from build123d import *

# Parameters (mm, degrees)
SKETCH_1_R          = 20
EXTRUDE_1_DEPTH     = 342.5
SKETCH_2_R          = 18
EXTRUDE_2_DEPTH     = 48
SKETCH_3_R          = 17.5
EXTRUDE_3_DEPTH     = 40
EXTRUDE_START       = 48
SKETCH_4_R          = 18
EXTRUDE_4_DEPTH     = 48
EXTRUDE_START_2     = 40
SKETCH_5_R          = 17.5
EXTRUDE_5_DEPTH     = 40
CUT_EXTRUDE_1_DEPTH = 5.71
CHAMFER_1_SIZE      = 2


with BuildPart() as part:
    # 草图1 → 凸台-拉伸1 (new, symmetric)
    with BuildSketch(Plane(origin=(0, 0, 0), x_dir=(0, 0, -1), z_dir=(1, 0, 0))):
        Circle(SKETCH_1_R)
    extrude(amount=EXTRUDE_1_DEPTH, both=True)

    # 草图2 → 凸台-拉伸2 (add)
    with BuildSketch(Plane.ZY.offset(342.5)):
        with Locations(Location((0, 0, 0), (0, 0, 180))):
            Circle(SKETCH_2_R)
    extrude(amount=EXTRUDE_2_DEPTH)

    # 草图3 → 凸台-拉伸3 (add)
    with BuildSketch(Plane.ZY.offset(390.5)):
        Circle(SKETCH_3_R)
    extrude(amount=EXTRUDE_3_DEPTH)

    # 草图4 → 凸台-拉伸4 (add)
    with BuildSketch(Plane(origin=(342.5, 0, 0), x_dir=(0, 0, -1), z_dir=(1, 0, 0)).offset(EXTRUDE_START)):
        Circle(SKETCH_4_R)
    extrude(amount=-EXTRUDE_4_DEPTH)

    # 草图5 → 凸台-拉伸5 (add)
    with BuildSketch(Plane(origin=(390.5, 0, 0), x_dir=(0, 0, -1), z_dir=(1, 0, 0)).offset(EXTRUDE_START_2)):
        with Locations(Location((0, 0, 0), (0, 0, 180))):
            Circle(SKETCH_5_R)
    extrude(amount=-EXTRUDE_5_DEPTH)

    # 草图7 → 切除-拉伸1 (cut)
    with BuildSketch(Plane(origin=(0, 18, 0), x_dir=(1, 0, 0), z_dir=(0, 1, 0))):
        with BuildLine():
            Line((351.5, 5), (381.5, 5))
            ThreePointArc((381.5, 5), (386.5, 0), (381.5, -5))
            Line((381.5, -5), (351.5, -5))
            ThreePointArc((351.5, -5), (346.5, 0), (351.5, 5))
        make_face()
        with BuildLine():
            Line((-351.5, -5), (-381.5, -5))
            ThreePointArc((-381.5, -5), (-386.5, 0), (-381.5, 5))
            Line((-381.5, 5), (-351.5, 5))
            ThreePointArc((-351.5, 5), (-346.5, 0), (-351.5, -5))
        make_face()
    extrude(amount=-CUT_EXTRUDE_1_DEPTH, mode=Mode.SUBTRACT)

    # 倒角1
    chamfer_1_edges = [part.edges().sort_by_distance(p)[0] for p in [
        (-430.5, 0, -17.5),
        (430.5, 0, -17.5),
    ]]
    chamfer(chamfer_1_edges, length=CHAMFER_1_SIZE)


solid = part.part
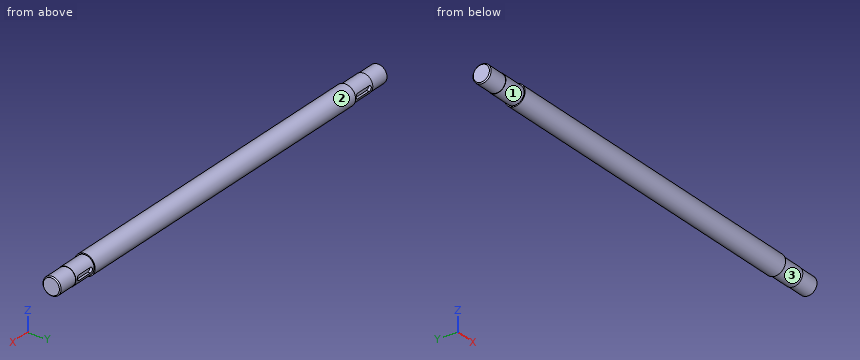
Verification items for the finished model (mm, model axes). Face numbers are marked on the shaded views. A direction names the side the tool comes from. Give positions to 0.01 mm unless a question says otherwise; leave off trailing zeros. Write each loop counter-clockwise with the first axis right and the second up, starting at its lowest first coordinate (ties: lowest second). Pieces come first, ordered by that corner, then holes.
(1) Gauge pin test, flat ends, axial feed: pin 1 (5 mm diameter, centred on x = 372, z = -2, fed in from +Y); pin 2 (1.5 mm diameter, centred on x = 211, z = -9.5, fed in from +Y); pin 3 (4 mm diameter, centred on x = -366.5, y = 15, fed in from +Z). Record the tip position at first contact, or that the pin passes through.
(2) Access from +Z, -Z, +X, -X, +Y, -Y to the whole of each face (thin tool, end or side, straight path). Record for the marked faces 1, 2 and 3.
(3) Cross-section at A-A (y = 0). Enter the section's corners in (x, z), plus the area to 3 significant figures.
(4) Cross-section at B-B (x = 303). Enter the section's corners in (y, z).
(5) Material ranges on line 1 (X direction, y = -14, z = -13.5); line 2 (Y direction, x = 384, z = 4.5); line 3 (Z direction, x = 316, y = 0.5), recorded low to high.
Worked out:
1. pin 1: stops at y = 12.29
1. pin 2: stops at y = 17.98
1. pin 3: stops at z = 12.45
2. face 1: -X
2. face 2: +X, -X
2. face 3: +X
3. outline: (-430.5, -15.5) - (-428.5, -17.5) - (-390.5, -17.5) - (-390.5, -18) - (-342.5, -18) - (-342.5, -20) - (342.5, -20) - (342.5, -18) - (390.5, -18) - (390.5, -17.5) - (428.5, -17.5) - (430.5, -15.5) - (430.5, 15.5) - (428.5, 17.5) - (390.5, 17.5) - (390.5, 18) - (342.5, 18) - (342.5, 20) - (-342.5, 20) - (-342.5, 18) - (-390.5, 18) - (-390.5, 17.5) - (-428.5, 17.5) - (-430.5, 15.5) - close
3. area: 33,600 mm2
4. outline: circle Ø40 at (0, 0)
5. line 1: x = -342.5 to 342.5
5. line 2: y = -17.43 to 17.43
5. line 3: z = -19.99 to 19.99
